```python
from build123d import *

# Parameters (mm, degrees)
SKETCH1_W                 = 50
SKETCH1_H                 = 50
BOSS_EXTRUDE1_DEPTH       = 45
SKETCH3_R                 = 12.5
CUT_EXTRUDE1_DEPTH        = 56
CHAMFER1_SIZE             = 15
M8X1_0_TAPPED_HOLE1_D     = 7
M8X1_0_TAPPED_HOLE1_DEPTH = 19
M8X1_0_TAPPED_HOLE1_TIP   = 2.103012167
CHAMFER2_SIZE             = 0.2
CHAMFER3_SIZE             = 0.2


with BuildPart() as part:
    # Sketch1 → Boss-Extrude1 (new body)
    with BuildSketch(Plane.XY):
        Rectangle(SKETCH1_W, SKETCH1_H)
    extrude(amount=BOSS_EXTRUDE1_DEPTH)

    # Sketch3 → Cut-Extrude1 (cut)
    with BuildSketch(Plane(origin=(25, 0, 0), x_dir=(0, 0, -1), z_dir=(1, 0, 0))):
        with Locations(Location((-27, 0, 0), (0, 0, 90))):
            Circle(SKETCH3_R)
    extrude(amount=-CUT_EXTRUDE1_DEPTH, mode=Mode.SUBTRACT)

    # Chamfer1
    chamfer1_edges = [part.edges().sort_by_distance(p)[0] for p in [
        (0, -25, 45),
        (0, 25, 45),
    ]]
    chamfer(chamfer1_edges, length=CHAMFER1_SIZE)

    # M8x1.0 Tapped Hole1
    with Locations(Plane(origin=(0, 0, 0), x_dir=(-1, 0, 0), z_dir=(0, 0, -1))):
        with Locations((-18, 18.5), (18, 18.5), (18, -18.5), (-18, -18.5)):
            Hole(M8X1_0_TAPPED_HOLE1_D / 2, depth=M8X1_0_TAPPED_HOLE1_DEPTH)
            with Locations((0, 0, -(M8X1_0_TAPPED_HOLE1_DEPTH + M8X1_0_TAPPED_HOLE1_TIP / 2))):  # 118° drill point
                Cone(0, M8X1_0_TAPPED_HOLE1_D / 2, M8X1_0_TAPPED_HOLE1_TIP, mode=Mode.SUBTRACT)

    # Chamfer2
    chamfer2_edges = [part.edges().sort_by_distance(p)[0] for p in [
        (25, -12.5, 27),
    ]]
    chamfer(chamfer2_edges, length=CHAMFER2_SIZE)

    # Chamfer3
    chamfer3_edges = [part.edges().sort_by_distance(p)[0] for p in [
        (-25, -12.5, 27),
    ]]
    chamfer(chamfer3_edges, length=CHAMFER3_SIZE)


solid = part.part
```
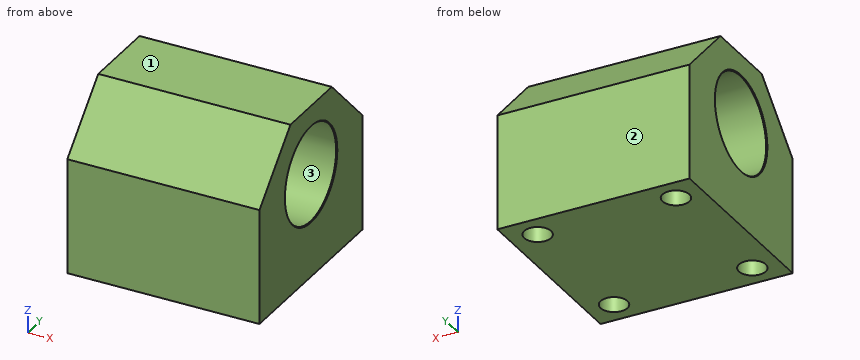
Geometry: final body of the model. Coordinates: model frame, mm. Face numbers are marked on the shaded views. Round coordinates to 2 decimals unless told otherwise and drop trailing zeros. Write each loop counter-clockwise with the first axis right and the second up, starting at its lowest first coordinate (ties: lowest second). Pieces come first, ordered by that corner, then holes. Notation, with made-up numbers: M -37.75,36 L -8.75,36 A15 cw -8.75,60 Z; hole C 40.25,42 d5. An arc over 180 degrees is marked long. Answer in a Markdown table with one row per item. Add a question column.
(1) Ray query, L1, parallel to X at y = -18.5, z = 13.25; L2, parallel to Y at x = 18, z = 9.5; L3, parallel to Y at x = -20, z = 13. Return the intervals inside material, ascending.
(2) Draft query along Z for the marked faces 1, 2 and 3. Return one class per face: pulls with the +Z half, pulls with the -Z half, needs draft (parallel to the pull), parting line crosses it, or undercut.
(3) Cut plane B-B, the plane x = -1.5. Return the cut outline in (y, z), then the cut area to 3 significant figures.
(4) Cut plane A-A, the plane y = 0. Return the cut outline in (x, z).
(5) Cut plane D-D, the plane z = 12. Return the cut outline in (x, y), then the cut area to 3 significant figures.
(6) Cut plane C-C, the plane z = 27. Return the cut outline in (x, y).
(7) Contact query for flat-ended pins moving along their axis: pin 1 (1.5 mm diameter, centred on x = 12.5, y = 12, fed in from +Z); pin 2 (4 mm diameter, centred on x = -18, y = -18.5, fed in from -Z); pin 3 (6.5 mm diameter, centred on x = 18, y = -18.5, fed in from +Z). Output: stop coordinate, or through.
Established:
| question | item | result |
|---|---|---|
| 1 | L1 | -25 to -21.5, -14.5 to 14.5, 21.5 to 25 |
| 1 | L2 | -25 to -22, -15 to 15, 22 to 25 |
| 1 | L3 | -25 to -21.37, -15.63 to 15.63, 21.37 to 25 |
| 2 | face 1 | pulls with the +Z half |
| 2 | face 2 | needs draft |
| 2 | face 3 | undercut |
| 3 | outline | M -25,0 L 25,0 L 25,30 L 10,45 L -10,45 L -25,30 Z; hole C 0,27 d25 |
| 3 | area | 1,530 mm² |
| 4 | outline | M -25,0 L 25,0 L 25,14.3 L 24.8,14.5 L -24.8,14.5 L -25,14.3 Z; M -25,39.7 L -24.8,39.5 L 24.8,39.5 L 25,39.7 L 25,45 L -25,45 Z |
| 5 | outline | M -25,-25 L 25,-25 L 25,25 L -25,25 Z; hole C -18,-18.5 d7; hole C -18,18.5 d7; hole C 18,-18.5 d7; hole C 18,18.5 d7 |
| 5 | area | 2,350 mm² |
| 6 | outline | M -25,-25 L 25,-25 L 25,-12.7 L 24.8,-12.5 L -24.8,-12.5 L -25,-12.7 Z; M -25,12.7 L -24.8,12.5 L 24.8,12.5 L 25,12.7 L 25,25 L -25,25 Z |
| 7 | pin 1 | z = 43.75 |
| 7 | pin 2 | z = 19.9 |
| 7 | pin 3 | z = 39.75 |
